Read the model definition and answer for the solid it produces. Units are mm, in the model's axes. Coordinates: 2 decimals unless noted, no trailing zeros. Write each loop counter-clockwise with the first axis right and the second up, starting at its lowest first coordinate (ties: lowest second). Pieces come first, ordered by that corner, then holes.
(1) The mould has two halves that part along X. Classify faces 1 (the cylindrical face through (94.84, 137.59, 7.89)), 2 (the flat face through (-2, 2, 0)), 3 (the flat face through (-120, -2, 8)), 4 (the cylindrical face through (-85.16, 137.59, 7.89)): +X half, -X half, draft (parallel to the pull), parting line (faces both ways), or undercut.
(2) Section A-A on y = -130 is taken. Write down the section's boundary in (x, z), then the cut area to 3 significant figures.
(3) Given pin 1 (23.5 mm diameter, centred on x = 90, y = 130, fed in from -Z), flat-ended and moving along its own axis, determine where the tip first touches the part or whether it passes through.
(4) Section B-B on x = -90 is taken. Write down the section's boundary in (y, z).
(5) Find the intervals of material crossed by probe 1 along Y at (x, z) = (90, 3.5), in increasing order.
from build123d import *

# Parameters (mm, degrees)
SKETCH2_W           = 240
SKETCH2_H           = 340
SKETCH2_R           = 9
BOSS_EXTRUDE1_DEPTH = 16


with BuildPart() as part:
    # Sketch2 → Boss-Extrude1 (new body)
    with BuildSketch(Plane.XY):
        Rectangle(SKETCH2_W, SKETCH2_H)
        with Locations((-90, 130)):
            Circle(SKETCH2_R, mode=Mode.SUBTRACT)
        with Locations((90, 130)):
            Circle(SKETCH2_R, mode=Mode.SUBTRACT)
        with Locations((90, -130)):
            Circle(SKETCH2_R, mode=Mode.SUBTRACT)
        with Locations((-90, -130)):
            Circle(SKETCH2_R, mode=Mode.SUBTRACT)
    extrude(amount=BOSS_EXTRUDE1_DEPTH)


solid = part.part
Response:
1. face 1: undercut
1. face 2: draft
1. face 3: -X half
1. face 4: undercut
2. outline: (-120, 0) - (-99, 0) - (-99, 16) - (-120, 16) - close; (-81, 0) - (81, 0) - (81, 16) - (-81, 16) - close; (99, 0) - (120, 0) - (120, 16) - (99, 16) - close
2. area: 3,260 mm2
3. pin 1: stops at z = 0
4. outline: (-170, 0) - (-139, 0) - (-139, 16) - (-170, 16) - close; (-121, 0) - (121, 0) - (121, 16) - (-121, 16) - close; (139, 0) - (170, 0) - (170, 16) - (139, 16) - close
5. probe 1: y = -170 to -139, -121 to 121, 139 to 170
